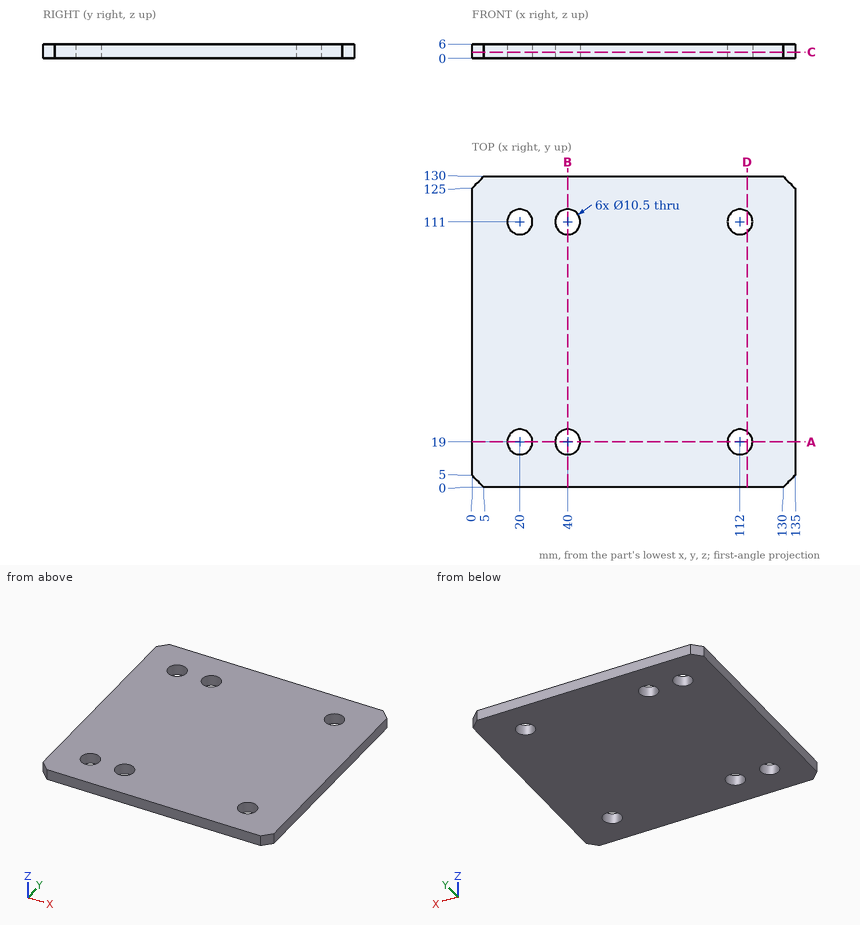
The drawing under review shows one solid part. Ordinate dimensions are in mm from its lowest x, y, z. Round coordinates to 2 decimals unless told otherwise and drop trailing zeros. Loops run counter-clockwise (first coordinate to the right, second up) from the corner with the lowest first, then second, coordinate; pieces in that order, holes last. Notation, with made-up numbers: (-7, 27.25) -> (24, 27.25) arc R16 cw to (24, 48.25) -> close; hole circle Ø7 at (4.25, 15.25). An arc over 180 degrees is marked (long way). One line per question, with ' | ' between items. Start each with the question number.
Item 1: Add section C-C, the plane z = 2.6. Write out the cut boundary in (x, y), then the cut area to 3 significant figures.
Item 2: Wall thickness on line 1 along X through (y, z) = (19, 2.8); line 2 along Y through (x, z) = (40, 4.45); line 3 along Y through (x, z) = (23, 1.35): over which ranges is each line inside the solid? List them lowest first. Write a range as [from, to].
Item 3: Add section D-D, the plane x = 115. Write out the cut boundary in (y, z), then the cut area to 3 significant figures.
Item 4: Add section B-B, the plane x = 40. Write out the cut boundary in (y, z), then the cut area to 3 significant figures.
Item 5: Add section A-A, the plane y = 19. Write out the cut boundary in (x, z), then the cut area to 3 significant figures.
Return value:
1) outline: (0, 5) -> (5, 0) -> (130, 0) -> (135, 5) -> (135, 125) -> (130, 130) -> (5, 130) -> (0, 125) -> close; hole circle Ø10.5 at (20, 19); hole circle Ø10.5 at (20, 111); hole circle Ø10.5 at (40, 19); hole circle Ø10.5 at (40, 111); hole circle Ø10.5 at (112, 19); hole circle Ø10.5 at (112, 111) | area: 17,000 mm2
2) line 1: x = [0, 14.75], [25.25, 34.75], [45.25, 106.75], [117.25, 135] | line 2: y = [0, 13.75], [24.25, 105.75], [116.25, 130] | line 3: y = [0, 14.69], [23.31, 106.69], [115.31, 130]
3) outline: (0, 0) -> (14.69, 0) -> (14.69, 6) -> (0, 6) -> close; (23.31, 0) -> (106.69, 0) -> (106.69, 6) -> (23.31, 6) -> close; (115.31, 0) -> (130, 0) -> (130, 6) -> (115.31, 6) -> close | area: 677 mm2
4) outline: (0, 0) -> (13.75, 0) -> (13.75, 6) -> (0, 6) -> close; (24.25, 0) -> (105.75, 0) -> (105.75, 6) -> (24.25, 6) -> close; (116.25, 0) -> (130, 0) -> (130, 6) -> (116.25, 6) -> close | area: 654 mm2
5) outline: (0, 0) -> (14.75, 0) -> (14.75, 6) -> (0, 6) -> close; (25.25, 0) -> (34.75, 0) -> (34.75, 6) -> (25.25, 6) -> close; (45.25, 0) -> (106.75, 0) -> (106.75, 6) -> (45.25, 6) -> close; (117.25, 0) -> (135, 0) -> (135, 6) -> (117.25, 6) -> close | area: 621 mm2
